```python
from build123d import *

# Parameters (mm, degrees)
BOSS_EXTRUDE1_DEPTH = 9


with BuildPart() as part:
    # Sketch1 → Boss-Extrude1 (new body)
    with BuildSketch(Plane.XY):
        with BuildLine():
            Line((0, 0), (-34, 0))
            Line((-34, 0), (-34, 19.555773208))
            ThreePointArc((-34, 19.555773208), (-33.980382319, 19.99825706), (-33.921683216, 20.437268709))
            Line((-33.921683216, 20.437268709), (-22.737642597, 82.881495501))
            ThreePointArc((-22.737642597, 82.881495501), (-21.024738159, 85.834545443), (-17.815959381, 87))
            Line((-17.815959381, 87), (-5, 87))
            ThreePointArc((-5, 87), (-1.464466094, 85.535533906), (0, 82))
            Line((0, 82), (0, 0))
        make_face()
    extrude(amount=BOSS_EXTRUDE1_DEPTH)


solid = part.part
```
Input: part model. Units: mm. Frame: model coordinates. Round coordinates to 2 decimals unless told otherwise and drop trailing zeros. Loops run counter-clockwise (first coordinate to the right, second up) from the corner with the lowest first, then second, coordinate; pieces in that order, holes last. Notation, with made-up numbers: (54.5, 2) -> (110.5, 2) arc R25 ccw to (110.5, 27) -> close; hole circle Ø3 at (51, -5.5). An arc over 180 degrees is marked (long way). Use one line per item in the form item = value. Start each with the question number.
Item 1: Section query B-B on x = -25. Return the cut outline in (y, z), then the cut area to 3 significant figures.
Item 2: Section query A-A on z = 5. Return the cut outline in (x, y), then the cut area to 3 significant figures.
Item 3: Material intervals for L1, parallel to X at y = 29, z = 5; L2, parallel to Y at x = -22, z = 4.25; L3, parallel to Y at x = -3, z = 6.25, sorted ascending. Write a range as from..to.
Item 4: Section query C-C on y = 41. Return the cut outline in (x, z).
Item 5: Contact query for a flat-ended pin moving along its axis: pin 1 Ø4 at (y, z) = (28, 8) entering from -X. Output: stop coordinate, or through.
Ans:
q1.outline = (0, 0) -> (70.25, 0) -> (70.25, 9) -> (0, 9) -> close
q1.area = 632 mm^2
q2.outline = (-34, 0) -> (0, 0) -> (0, 82) arc R5 ccw to (-5, 87) -> (-17.82, 87) arc R5 ccw to (-22.74, 82.88) -> (-33.92, 20.44) arc R5 ccw to (-34, 19.56) -> close
q2.area = 2,550 mm^2
q3.L1 = -32.39..0
q3.L2 = 0..84.74
q3.L3 = 0..86.58
q4.outline = (-30.24, 0) -> (0, 0) -> (0, 9) -> (-30.24, 9) -> close
q5.pin_1 = -32.93
